Could you check a few things on this model? Use its own coordinates, in mm. Round coordinates to 2 decimals unless told otherwise and drop trailing zeros. Loops run counter-clockwise (first coordinate to the right, second up) from the corner with the lowest first, then second, coordinate; pieces in that order, holes last. Notation, with made-up numbers: (-3, 29) -> (44, 29) arc R19 cw to (44, 36) -> close; hole circle Ø7 at (-39, 72). An arc over 180 degrees is marked (long way). Put each result on its own line as item: value. Start each with the question number.
1. I'm going to push flat-ended pins straight in: P1, Ø10, axis at x = 21.5, y = 24, coming from the +Z side; P2, Ø3, axis at y = 32.5, z = 33.5, coming from the +X side; P3, Ø10, axis at x = -5.5, y = 26.5, coming from the +Z side; P4, Ø1, axis at x = -32.5, z = -33, coming from the +Y side. Where does each tip first touch, or does it pass through?
2. Imagine slicing it at A-A, the plane x = 0. Please give me the cut outline in (y, z).
3. Imagine slicing it at C-C, the plane y = 44. Please give me the cut outline in (x, z).
4. Imagine slicing it at B-B, the plane z = 0. Please give me the cut outline in (x, y).
5. If we mould it in two halves opening along Z, with no side actions, what happens to faces 1 (the cylindrical face through (-21, 25, -28)), 2 (the flat face through (32, 50, 19)), 3 (the cylindrical face through (-17.235, 24.678, 41.569))? For each: pulls with the +Z half, pulls with the -Z half, needs draft (parallel to the pull), parting line crosses it, or undercut.
6. I need wall thicknesses on line 1 (X direction, y = 31, z = 0); line 2 (X direction, y = 25, z = 31); line 3 (Z direction, x = -27, y = 31.5). Which ranges of each line are inside material? Lowest first, please. Write a range as [from, to].
```python
from build123d import *

# Parameters (mm, degrees)
SKETCH1_R           = 45
SKETCH1_R_2         = 35
BOSS_EXTRUDE1_DEPTH = 50
CHAMFER2_SIZE       = 2


with BuildPart() as part:
    # Sketch1 → Boss-Extrude1 (new body)
    with BuildSketch(Plane(origin=(0, 0, 0), x_dir=(1, 0, 0), z_dir=(0, 1, 0))):
        with Locations(Location((0, 0, 0), (0, 0, 270))):
            Circle(SKETCH1_R)
        with Locations(Location((0, 0, 0), (0, 0, 270))):
            Circle(SKETCH1_R_2, mode=Mode.SUBTRACT)
    extrude(amount=BOSS_EXTRUDE1_DEPTH)

    # Chamfer2
    chamfer2_edges = [part.edges().sort_by_distance(p)[0] for p in [
        (0, 0, -45),
        (0, 50, -45),
        (0, 0, -35),
        (0, 50, -35),
    ]]
    chamfer(chamfer2_edges, length=CHAMFER2_SIZE)


solid = part.part
```
Entries:
1. P1: z = 41.87
1. P2: x = 31.64
1. P3: z = 45
1. P4: through
2. outline: (0, -43) -> (2, -45) -> (48, -45) -> (50, -43) -> (50, -37) -> (48, -35) -> (2, -35) -> (0, -37) -> close; (0, 37) -> (2, 35) -> (48, 35) -> (50, 37) -> (50, 43) -> (48, 45) -> (2, 45) -> (0, 43) -> close
3. outline: circle Ø90 at (0, 0); hole circle Ø70 at (0, 0)
4. outline: (-45, 2) -> (-43, 0) -> (-37, 0) -> (-35, 2) -> (-35, 48) -> (-37, 50) -> (-43, 50) -> (-45, 48) -> close; (35, 2) -> (37, 0) -> (43, 0) -> (45, 2) -> (45, 48) -> (43, 50) -> (37, 50) -> (35, 48) -> close
5. face 1: undercut
5. face 2: needs draft
5. face 3: parting line crosses it
6. line 1: [-45, -35], [35, 45]
6. line 2: [-32.62, -16.25], [16.25, 32.62]
6. line 3: [-36, -22.27], [22.27, 36]
